```python
from build123d import *

# Parameters (mm, degrees)
BEARING_HOUSING_SKETCH_R   = 57.5
BEARING_HOUSING_SKETCH_R_2 = 37.5
BEARING_HOUSING_DEPTH      = 60
BRACKET_BODY_DEPTH         = 55
LOWER_BOSS_SKETCH_R        = 37.5
LOWER_BOSS_SKETCH_R_2      = 22.5
LOWER_BOSS_DEPTH           = 25
ANGLED_WEB_DEPTH           = 13
SIDE_LUG_DEPTH             = 30
SIDE_BOSS_SKETCH_R         = 30
SIDE_BOSS_SKETCH_R_2       = 12.5
SIDE_BOSS_DEPTH            = 6


with BuildPart() as part:
    # Bearing Housing Sketch → Bearing Housing (new, symmetric)
    with BuildSketch(Plane(origin=(0, 0, 0), x_dir=(0, 0, -1), z_dir=(1, 0, 0))):
        Circle(BEARING_HOUSING_SKETCH_R)
        Circle(BEARING_HOUSING_SKETCH_R_2, mode=Mode.SUBTRACT)
    extrude(amount=BEARING_HOUSING_DEPTH, both=True)

    # Bracket Body Sketch → Bracket Body (add, symmetric)
    with BuildSketch(Plane(origin=(0, 0, 0), x_dir=(0, 0, -1), z_dir=(1, 0, 0))):
        with BuildLine():
            Line((-57.5, 0), (-57.5, -165))
            Line((-57.5, -165), (0, -165))
            Line((0, -165), (0, -159))
            Line((0, -159), (75, -159))
            Line((75, -159), (75, -129))
            Line((75, -129), (-27.5, -129))
            Line((-27.5, -129), (-27.5, -50.497524692))
            ThreePointArc((-27.5, -50.497524692), (-49.434299833, -29.368350311), (-57.5, 0))
        make_face()
    extrude(amount=BRACKET_BODY_DEPTH, both=True)



with BuildPart() as body_2:
    # Lower Boss Sketch → Lower Boss (new, symmetric)
    with BuildSketch(Plane(origin=(0, 0, 0), x_dir=(0, 0, -1), z_dir=(1, 0, 0))):
        with Locations((-110, -90)):
            Circle(LOWER_BOSS_SKETCH_R)
        with Locations((-110, -90)):
            Circle(LOWER_BOSS_SKETCH_R_2, mode=Mode.SUBTRACT)
    extrude(amount=LOWER_BOSS_DEPTH, both=True)


with BuildPart() as part_1:
    add(part.part)

    add(body_2.part)  # Angled Web merges body 2
    # Angled Web Sketch → Angled Web (add, symmetric)
    with BuildSketch(Plane(origin=(0, 0, 0), x_dir=(0, 0, -1), z_dir=(1, 0, 0))):
        with BuildLine():
            Line((-57.5, 0), (-57.5, -165))
            Line((-57.5, -165), (-129.216934712, -122.201854299))
            ThreePointArc((-129.216934712, -122.201854299), (-72.890500848, -84.60230858), (-137.594286915, -64.606982659))
            Line((-137.594286915, -64.606982659), (-42.311239936, 38.935959922))
            ThreePointArc((-42.311239936, 38.935959922), (-53.568396916, 20.896814394), (-57.5, 0))
        make_face()
    extrude(amount=ANGLED_WEB_DEPTH, both=True)

    # Side Lug Sketch → Side Lug (add)
    with BuildSketch(Plane(origin=(0, -129, 0), x_dir=(1, 0, 0), z_dir=(0, 1, 0))):
        with BuildLine():
            Line((-60, 111), (60, 111))
            ThreePointArc((60, 111), (95.912665801, 72.493920376), (55, 39.34891306))
            Line((55, 39.34891306), (55, -27.5))
            Line((55, -27.5), (-55, -27.5))
            Line((-55, -27.5), (-55, 39.34891306))
            ThreePointArc((-55, 39.34891306), (-95.912665801, 72.493920376), (-60, 111))
        make_face()
    extrude(amount=-SIDE_LUG_DEPTH)

    # Side Boss Sketch → Side Boss (add)
    # profile 1 of 2: a face of its own
    with BuildSketch(Plane(origin=(0, -129, 0), x_dir=(1, 0, 0), z_dir=(0, 1, 0))):
        with Locations(Location((60, 75, 0), (0, 0, 90))):
            Circle(SIDE_BOSS_SKETCH_R)
        with Locations(Location((60, 75, 0), (0, 0, 270))):
            Circle(SIDE_BOSS_SKETCH_R_2, mode=Mode.SUBTRACT)
    # profile 2 of 2: a face of its own
    with BuildSketch(Plane(origin=(0, -129, 0), x_dir=(1, 0, 0), z_dir=(0, 1, 0))):
        with Locations(Location((-60, 75, 0), (0, 0, 90))):
            Circle(SIDE_BOSS_SKETCH_R)
        with Locations(Location((-60, 75, 0), (0, 0, 270))):
            Circle(SIDE_BOSS_SKETCH_R_2, mode=Mode.SUBTRACT)
    extrude(amount=SIDE_BOSS_DEPTH)


solid = part_1.part
```
Work out the finished part from the listing and answer in its coordinate system (mm). A direction names the side the tool comes from. Round coordinates to 2 decimals unless told otherwise and drop trailing zeros. Order: outer loops, then holes, each group sorted by start corner. A loop starts at its lowest first (then second) coordinate and runs counter-clockwise, first axis right, second up.
Q1. Given pin 1 Ø22.5 at (y, z) = (-77.5, 102.5) entering from +X; pin 2 Ø6 at (x, z) = (57.5, -82) entering from +Y; pin 3 Ø1.5 at (x, y) = (39.5, -132.5) entering from +Z, each flat-ended and moving along its own axis, determine where each tip first touches the part or whether it passes through.
Solution:
pin 1: stops at x = 25
pin 2: stops at y = -129
pin 3: stops at z = 57.5
Q2. A cutting plane is placed at A-A, the plane x = 20.5. Determine the outline of the cut face in (y, z), then the cut area to 3 significant figures.
Solution:
outline: (-165, 0) - (-159, 0) - (-159, -111) - (-129, -111) - (-129, 27.5) - (-50.5, 27.5) arc R57.5 ccw (long way) to (0, 57.5) - (-165, 57.5) - close; circle Ø75 at (-90, 110); hole circle Ø45 at (-90, 110); hole circle Ø75 at (0, 0)
area: 17,000 mm2
Q3. A cutting plane is placed at B-B, the plane z = 110. Determine the outline of the cut face in (x, y).
Solution:
outline: (-25, -127.5) - (-13, -127.5) - (-13, -133.67) - (13, -133.67) - (13, -127.5) - (25, -127.5) - (25, -112.5) - (-25, -112.5) - close; (-25, -67.5) - (25, -67.5) - (25, -52.5) - (13, -52.5) - (13, -34.62) - (-13, -34.62) - (-13, -52.5) - (-25, -52.5) - close
Q4. A cutting plane is placed at D-D, the plane z = -75. Determine the outline of the cut face in (x, y), then the cut area to 3 significant figures.
Solution:
outline: (-96, -159) - (96, -159) - (96, -129) - (90, -129) - (90, -123) - (72.5, -123) - (72.5, -129) - (47.5, -129) - (47.5, -123) - (30, -123) - (30, -129) - (-30, -129) - (-30, -123) - (-47.5, -123) - (-47.5, -129) - (-72.5, -129) - (-72.5, -123) - (-90, -123) - (-90, -129) - (-96, -129) - close
area: 6,180 mm2
Q5. Find the intervals of material crossed by line 1 along X through (y, z) = (-125.8, -75); line 2 along Y through (x, z) = (-47.5, -49); line 3 along Y through (x, z) = (-37, -16), in increasing order.
Solution:
line 1: x = -90 to -72.5, -47.5 to -30, 30 to 47.5, 72.5 to 90
line 2: y = -159 to -123, -30.09 to 30.09
line 3: y = -159 to -129, -55.23 to -33.92, 33.92 to 55.23
Q6. The mould has two halves that part along X. Classify faces 1 (the cylindrical face through (-61.32, -126.04, -45.03)), 2 (the flat face through (34, -81, 57.5)), 3 (the flat face through (25, -106.1, 93.9)): pulls with the +X half, pulls with the -X half, needs draft (parallel to the pull), parting line crosses it, or undercut.
Solution:
face 1: undercut
face 2: needs draft
face 3: pulls with the +X half
Q7. A cutting plane is placed at C-C, the plane y = 3.5. Determine the outline of the cut face in (x, z).
Solution:
outline: (-60, -57.39) - (60, -57.39) - (60, -37.34) - (-60, -37.34) - close; (-60, 37.34) - (60, 37.34) - (60, 57.39) - (13, 57.39) - (13, 74.92) - (-13, 74.92) - (-13, 57.39) - (-60, 57.39) - close
Q8. A tool of negligible diameter and unlimited length cuts with its end or side. For faces 4 (the flat face through (60, -38, 1)), 5 (the flat face through (1, -90, 27.5)), 6 (the cylindrical face through (-47.606, -126.042, -76.627)), 7 (the flat face through (1, -162, 0)), from which of +Z, -Z, +X, -X, +Y, -Y can it reach the whole face along a straight path? Write none if from no direction.
Solution:
face 4: +Z, -Z, +X, +Y
face 5: +X, -X
face 6: +Y
face 7: -Z, +X, -X, -Y
